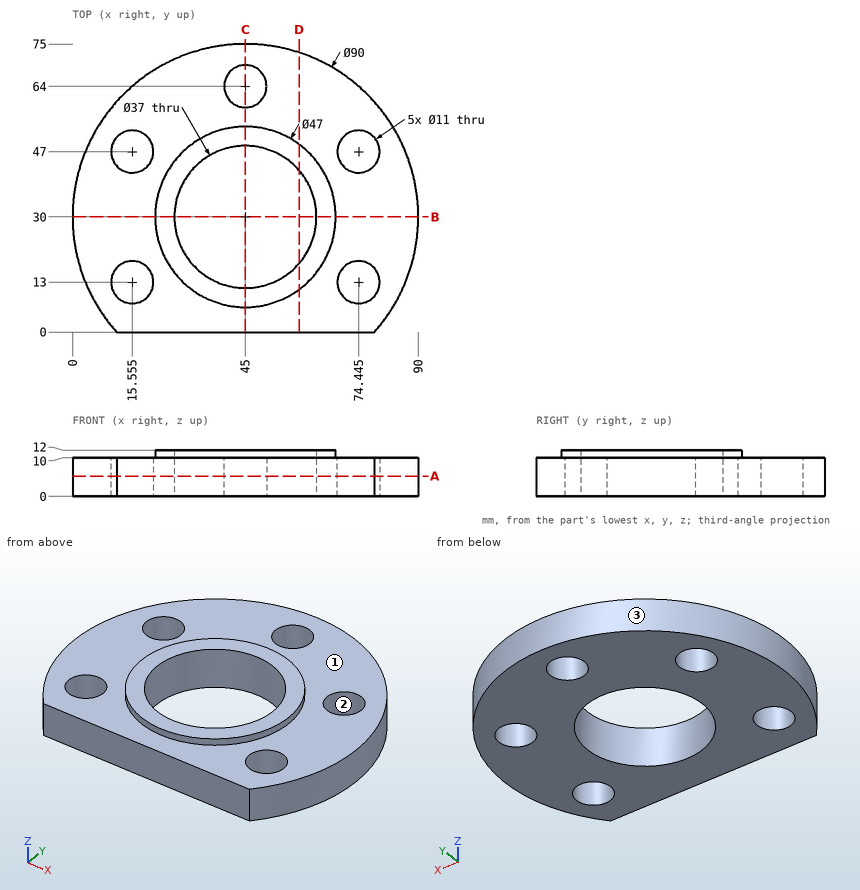
Geometry: see drawing. Coordinates: mm, zero at the bounding-box minimum. Give positions to 0.01 mm unless a question says otherwise; leave off trailing zeros. Order: outer loops, then holes, each group sorted by start corner. A loop starts at its lowest first (then second) coordinate and runs counter-clockwise, first axis right, second up. Notation, with made-up numbers: (-4.5, 2) - (37.5, 2) arc R24 cw to (37.5, 17) - close; hole circle Ø7 at (34.5, -28). An arc over 180 degrees is marked (long way). One line per item, written item: value.
1. Pin query (flat end, axial travel): pin 1 Ø12.5 at (x, y) = (45, 64) entering from +Z; pin 2 Ø6.5 at (x, y) = (74.44, 13) entering from +Z (3 decimals); pin 3 Ø2 at (y, z) = (8.5, 5) entering from -X; pin 4 Ø5 at (y, z) = (52.5, 2) entering from -X. Return the tip coordinate at first contact, or that it passes through.
Determined:
pin 1: z = 10
pin 2: through
pin 3: x = 4.94
pin 4: x = 4.69
2. Cut plane D-D, the plane x = 59. Output: boundary loops of the cut face in (y, z), and give its area (3 significant figures).
Determined:
outline: (0, 0) - (17.91, 0) - (17.91, 12) - (11.13, 12) - (11.13, 10) - (0, 10) - close; (42.09, 0) - (72.77, 0) - (72.77, 10) - (48.87, 10) - (48.87, 12) - (42.09, 12) - close
area: 513 mm2
3. Draft query along Y for the marked faces 1, 2 and 3. Return one class per face: released by +Y, released by -Y, zero draft, split by the parting line, or undercut.
Determined:
face 1: zero draft
face 2: undercut
face 3: split by the parting line
4. Cut plane A-A, the plane z = 5.25. Output: boundary loops of the cut face in (x, y) (3 decimals), and give its area (3 significant figures).
Determined:
outline: (11.459, 0) - (78.541, 0) arc R45 ccw (long way) to start; hole circle Ø11 at (15.555, 13); hole circle Ø11 at (15.555, 47); hole circle Ø37 at (45, 30); hole circle Ø11 at (45, 64); hole circle Ø11 at (74.445, 13); hole circle Ø11 at (74.445, 47)
area: 4,110 mm2
5. Line query: probe 1 along Y at (x, z) = (45.5, 4.5); probe 2 along Y at (x, z) = (46, 3.25); probe 3 along X at (y, z) = (43.5, 4.25). Output: solid intervals per line, ascending.
Determined:
probe 1: 0 to 11.51, 48.49 to 58.52, 69.48 to 75
probe 2: 0 to 11.53, 48.47 to 58.59, 69.41 to 74.99
probe 3: 2.07 to 11.31, 19.8 to 32.35, 57.65 to 70.2, 78.69 to 87.93
6. Cut plane C-C, the plane x = 45. Output: boundary loops of the cut face in (y, z).
Determined:
outline: (0, 0) - (11.5, 0) - (11.5, 12) - (6.5, 12) - (6.5, 10) - (0, 10) - close; (48.5, 0) - (58.5, 0) - (58.5, 10) - (53.5, 10) - (53.5, 12) - (48.5, 12) - close; (69.5, 0) - (75, 0) - (75, 10) - (69.5, 10) - close
7. Cut plane B-B, the plane y = 30. Output: boundary loops of the cut face in (x, z).
Determined:
outline: (0, 0) - (26.5, 0) - (26.5, 12) - (21.5, 12) - (21.5, 10) - (0, 10) - close; (63.5, 0) - (90, 0) - (90, 10) - (68.5, 10) - (68.5, 12) - (63.5, 12) - close
